from build123d import *

# Parameters (mm, degrees)
BASE_PLATE_DEPTH             = 10
MOUNTING_HOLES_2X_DEPTH      = 86.622718948
MOUNTING_HOLES_2X_DEPTH_BACK = 86.622718948
MOUNTING_HOLES_PROFILE_R     = 12.5
HUB_PROFILE_R                = 30.395167717
HUB_DEPTH                    = 60
BORE_PROFILE_35_R            = 17.5
BORE_35_DEPTH                = 60
CROSS_SLOTS_4X_DEPTH         = 5


with BuildPart() as part:
    # Base Plate Profile → Base Plate (new body)
    with BuildSketch(Plane(origin=(0, 0, 0), x_dir=(1, 0, 0), z_dir=(0, 1, 0))):
        with BuildLine():
            Line((19.30748114, -62.717391304), (33.788091995, -9.130434783))
            ThreePointArc((33.788091995, -9.130434783), (35, 0), (33.788091995, 9.130434783))
            Line((33.788091995, 9.130434783), (19.30748114, 62.717391304))
            ThreePointArc((19.30748114, 62.717391304), (0, 77.5), (-19.30748114, 62.717391304))
            Line((-19.30748114, 62.717391304), (-33.788091995, 9.130434783))
            ThreePointArc((-33.788091995, 9.130434783), (-35, 0), (-33.788091995, -9.130434783))
            Line((-33.788091995, -9.130434783), (-19.30748114, -62.717391304))
            ThreePointArc((-19.30748114, -62.717391304), (0, -77.5), (19.30748114, -62.717391304))
        make_face()
    extrude(amount=BASE_PLATE_DEPTH)

    # Mounting Holes Profile → Mounting Holes 2x (cut, two sides: drawn at the far end of the back side and taken through both)
    with BuildSketch(Plane(origin=(0, 10, 0), x_dir=(1, 0, 0), z_dir=(0, 1, 0)).offset(-MOUNTING_HOLES_2X_DEPTH_BACK)):
        with Locations(Location((0, 57.5, 0), (0, 0, 270))):
            Circle(MOUNTING_HOLES_PROFILE_R)
        with Locations(Location((0, -57.5, 0), (0, 0, 270))):
            Circle(MOUNTING_HOLES_PROFILE_R)
    extrude(amount=MOUNTING_HOLES_2X_DEPTH + MOUNTING_HOLES_2X_DEPTH_BACK, mode=Mode.SUBTRACT)

    # Hub Profile → Hub (add)
    with BuildSketch(Plane(origin=(0, 10, 0), x_dir=(1, 0, 0), z_dir=(0, 1, 0))):
        with Locations(Location((0, 0, 0), (0, 0, 270))):
            Circle(HUB_PROFILE_R)
    extrude(amount=HUB_DEPTH)

    # Bore Profile Ø35 → Bore Ø35 (cut)
    with BuildSketch(Plane(origin=(0, 70, 0), x_dir=(1, 0, 0), z_dir=(0, 1, 0))):
        with Locations(Location((0, 0, 0), (0, 0, 270))):
            Circle(BORE_PROFILE_35_R)
    extrude(amount=-BORE_35_DEPTH, mode=Mode.SUBTRACT)

    # Cross Slots Profile → Cross Slots 4x (cut)
    with BuildSketch(Plane(origin=(0, 70, 0), x_dir=(1, 0, 0), z_dir=(0, 1, 0))):
        with BuildLine():
            Line((-16.770509831, -5), (-29.981097721, -5))
            ThreePointArc((-29.981097721, -5), (-30.395167717, 0), (-29.981097721, 5))
            Line((-29.981097721, 5), (-16.770509831, 5))
            ThreePointArc((-16.770509831, 5), (-17.5, 0), (-16.770509831, -5))
        make_face()
        with BuildLine():
            Line((-5, -16.770509831), (-5, -29.981097721))
            ThreePointArc((-5, -29.981097721), (0, -30.395167717), (5, -29.981097721))
            Line((5, -29.981097721), (5, -16.770509831))
            ThreePointArc((5, -16.770509831), (0, -17.5), (-5, -16.770509831))
        make_face()
        with BuildLine():
            Line((-5, 16.770509831), (-5, 29.981097721))
            ThreePointArc((-5, 29.981097721), (0, 30.395167717), (5, 29.981097721))
            Line((5, 29.981097721), (5, 16.770509831))
            ThreePointArc((5, 16.770509831), (0, 17.5), (-5, 16.770509831))
        make_face()
        with BuildLine():
            Line((16.770509831, 5), (29.981097721, 5))
            ThreePointArc((29.981097721, 5), (30.395167717, 0), (29.981097721, -5))
            Line((29.981097721, -5), (16.770509831, -5))
            ThreePointArc((16.770509831, -5), (17.5, 0), (16.770509831, 5))
        make_face()
    extrude(amount=-CROSS_SLOTS_4X_DEPTH, mode=Mode.SUBTRACT)


solid = part.part
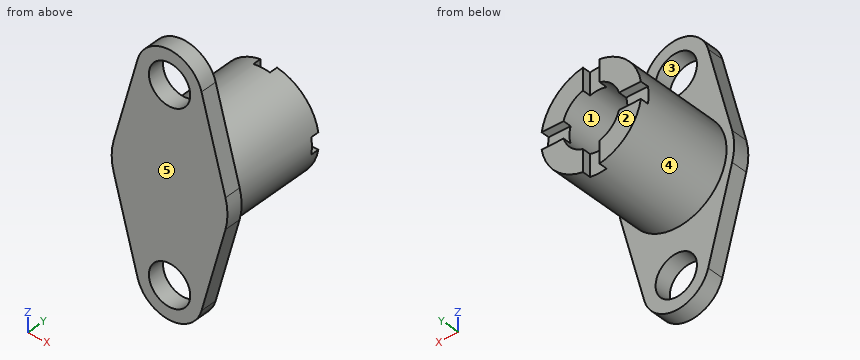
The listing builds one solid part. Answer for the finished solid, in the listing's coordinates (mm). Face numbers are marked on the shaded views. A direction names the side the tool comes from. Give positions to 0.01 mm unless a question says otherwise; leave off trailing zeros. Order: outer loops, then holes, each group sorted by start corner. A loop starts at its lowest first (then second) coordinate and runs counter-clockwise, first axis right, second up. Notation, with made-up numbers: (77, 8.25) - (95, 8.25) arc R19 cw to (95, 25.25) - close; hole circle Ø1 at (40, -30). An arc over 180 degrees is marked (long way). Use one line per item in the form item = value.
1) Each of these flat-tipped pins is pushed along its axis until it touches: pin 1 (10 mm diameter, centred on x = -10, y = 17.5, fed in from +Z); pin 2 (2.5 mm diameter, centred on x = -23.5, y = 68, fed in from -Z); pin 3 (1.5 mm diameter, centred on x = -0.5, y = 27, fed in from -Z). Where does it stop, or does it pass through?
Verdict:
pin_1 = 29.98
pin_2 = -20.71
pin_3 = -30.4
2) Find section B-B on x = 0. Determine the outline of the cut face in (y, z), and give its area (3 significant figures).
Verdict:
outline = (0, -77.5) - (10, -77.5) - (10, -70) - (0, -70) - close; (0, -45) - (10, -45) - (10, -30.4) - (65, -30.4) - (65, -17.5) - (10, -17.5) - (10, 17.5) - (65, 17.5) - (65, 30.4) - (10, 30.4) - (10, 45) - (0, 45) - close; (0, 70) - (10, 70) - (10, 77.5) - (0, 77.5) - close
area = 2,470 mm^2
3) The mould has two halves that part along X. Classify the marked faces 3, 4 and 5: released by +X, released by -X, zero draft, split by the parting line, or undercut.
Verdict:
face_3 = undercut
face_4 = split by the parting line
face_5 = zero draft
4) Find section C-C on z = -57.5. Determine the outline of the cut face in (x, y).
Verdict:
outline = (-20.72, 0) - (-12.5, 0) - (-12.5, 10) - (-20.72, 10) - close; (12.5, 0) - (20.72, 0) - (20.72, 10) - (12.5, 10) - close
5) Find section A-A on y = 5. Determine the outline of the cut face in (x, z), and give its area (3 significant figures).
Verdict:
outline = (-33.79, -9.13) - (-19.31, -62.72) arc R20 ccw to (19.31, -62.72) - (33.79, -9.13) arc R35 ccw to (33.79, 9.13) - (19.31, 62.72) arc R20 ccw to (-19.31, 62.72) - (-33.79, 9.13) arc R35 ccw to start; hole circle Ø25 at (0, -57.5); hole circle Ø25 at (0, 57.5)
area = 6,820 mm^2
6) Find section D-D on y = 20.5. Determine the outline of the cut face in (x, z), and give its area (3 significant figures).
Verdict:
outline = circle Ø60.79 at (0, 0); hole circle Ø35 at (0, 0)
area = 1,940 mm^2
7) For the marked faces 1 and 2, determine the directions among +Z, -Z, +X, -X, +Y, -Y from which every point of the face is accessible in a straight line to the end or side of a thin tool.
Verdict:
face_1 = +Y
face_2 = +Z, -Z, +X, -X, +Y
8) Consider probe 1 along X at (y, z) = (29, 0); probe 2 along Y at (x, z) = (-3, -16); probe 3 along Y at (x, z) = (3, -29.5). Determine where each line is inside the solid, lowest interval first. Write a range as [from, to].
Verdict:
probe_1 = [-30.4, -17.5], [17.5, 30.4]
probe_2 = [0, 10]
probe_3 = [0, 65]
